from build123d import *

# Parameters (mm, degrees)
SKETCH_1_R      = 10
SKETCH_1_R_2    = 5
EXTRUDE_1_DEPTH = 12.5
SKETCH_2_R      = 12.5
SKETCH_2_R_2    = 10
EXTRUDE_2_DEPTH = 10
CHAMFER_1_SIZE  = 1


with BuildPart() as part:
    # 草图1 → 凸台-拉伸1 (new, symmetric)
    with BuildSketch(Plane(origin=(0, 0, 0), x_dir=(0, 0, -1), z_dir=(1, 0, 0))):
        Circle(SKETCH_1_R)
        Circle(SKETCH_1_R_2, mode=Mode.SUBTRACT)
    extrude(amount=EXTRUDE_1_DEPTH, both=True)

    # 草图2 → 凸台-拉伸2 (add, symmetric)
    with BuildSketch(Plane(origin=(0, 0, 0), x_dir=(0, 0, -1), z_dir=(1, 0, 0))):
        Circle(SKETCH_2_R)
        Circle(SKETCH_2_R_2, mode=Mode.SUBTRACT)
    extrude(amount=EXTRUDE_2_DEPTH, both=True)

    # 倒角1
    chamfer_1_edges = [part.edges().sort_by_distance(p)[0] for p in [
        (-12.5, 0, 10),
        (12.5, 0, 10),
    ]]
    chamfer(chamfer_1_edges, length=CHAMFER_1_SIZE)


solid = part.part
Work out the finished part from the listing and answer in its coordinate system (mm). A direction names the side the tool comes from. Give positions to 0.01 mm unless a question says otherwise; leave off trailing zeros. Loops run counter-clockwise (first coordinate to the right, second up) from the corner with the lowest first, then second, coordinate; pieces in that order, holes last. Notation, with made-up numbers: M 17,42 L 70,42 A25 cw 70,56 Z; hole C 34.25,-20 d10. An arc over 180 degrees is marked long. Use CSV: the item, a comma, the result in double quotes.
1) Consider L1, parallel to Y at x = 3.75, z = 0; L2, parallel to X at y = 10.75, z = 5; L3, parallel to Z at x = 9, y = -1.75. Determine where each line is inside the solid, lowest interval first.
Answer:
L1,"-12.5 to -5, 5 to 12.5"
L2,"-10 to 10"
L3,"-12.38 to -4.68, 4.68 to 12.38"
2) Find section A-A on z = 0. Write down the section's boundary in (x, y).
Answer:
outline,"M -12.5,-9 L -11.5,-10 L -10,-10 L -10,-12.5 L 10,-12.5 L 10,-10 L 11.5,-10 L 12.5,-9 L 12.5,-5 L -12.5,-5 Z; M -12.5,5 L 12.5,5 L 12.5,9 L 11.5,10 L 10,10 L 10,12.5 L -10,12.5 L -10,10 L -11.5,10 L -12.5,9 Z"
3) Determine the mould class of faces 4 (the cylindrical face through (-0.18, -4.88, 1.08)), 5 (the cylindrical face through (10.76, -9.76, 2.17)), 6 (the flat face through (-12.5, -4, -4)) for opening direction Z: released by +Z, released by -Z, zero draft, split by the parting line, or undercut.
Answer:
face 4,"undercut"
face 5,"split by the parting line"
face 6,"zero draft"
4) Find section C-C on x = -4.5. Write down the section's boundary in (y, z), plus the area to 3 significant figures.
Answer:
outline,"C 0,0 d25; hole C 0,0 d10"
area,"412 mm^2"
5) Which of the six approach directions +Z, -Z, +X, -X, +Y, -Y give full straight-line access (tool end or side, diameter ignored) to faces 1 (the cylindrical face through (-10.74, -9.76, 2.17)), 2 (the flat face through (12.5, -4, -4)), 3 (the flat face through (10, 10.2, 0.1))?
Answer:
face 1,"-X"
face 2,"+Z, -Z, +X, +Y, -Y"
face 3,"+X"
6) Given P1, Ø3, axis at x = -0.5, z = -6.5, coming from the -Y side; P2, Ø4, axis at x = -2.5, z = -3.5, coming from the +Y side; P3, Ø12, axis at x = -7, y = 9.5, coming from the +Z side, each flat-ended and moving along its own axis, determine where each tip first touches the part or whether it passes through.
Answer:
P1,"y = -11.46"
P2,"y = 12.41"
P3,"z = 12"
7) Find section D-D on z = 11. Write down the section's boundary in (x, y), plus the area to 3 significant figures.
Answer:
outline,"M -10,-5.94 L 10,-5.94 L 10,5.94 L -10,5.94 Z"
area,"237 mm^2"
